from build123d import *

# Parameters (mm, degrees)
SKETCH_1_W      = 8
SKETCH_1_H      = 26
EXTRUDE_1_DEPTH = 525


with BuildPart() as part:
    # 草图1 → 凸台-拉伸1 (new, symmetric)
    with BuildSketch(Plane.XY):
        Polygon((-12, 4.5), (-10, 4.5), (-10, 6.5), (-4, 6.5), (-4, -6.5), (-10, -6.5), (-10, -4.5), (-12, -4.5), (-12, -36.5), (0, -36.5), (0, 36.5), (-12, 36.5), align=None)
        with Locations((-6, -21.5)):
            Rectangle(SKETCH_1_W, SKETCH_1_H, mode=Mode.SUBTRACT)
        with Locations((-6, 21.5)):
            Rectangle(SKETCH_1_W, SKETCH_1_H, mode=Mode.SUBTRACT)
    extrude(amount=EXTRUDE_1_DEPTH, both=True)


solid = part.part
Here's how the part is built. I have some questions about the finished solid (model axes, mm). A direction names the side the tool comes from. Give positions to 0.01 mm unless a question says otherwise; leave off trailing zeros. Order: outer loops, then holes, each group sorted by start corner. A loop starts at its lowest first (then second) coordinate and runs counter-clockwise, first axis right, second up. Notation, with made-up numbers: (-24, 78.25) -> (27, 78.25) arc R30 ccw to (27, 100.25) -> close; hole circle Ø8 at (57.5, 24). An arc over 180 degrees is marked (long way). Use a Markdown table: item, result. Add a question column.
Item 1: Imagine slicing it at C-C on z = 237. Please give me the cut outline in (x, y), plus the area to 3 significant figures.
Item 2: Imagine slicing it at B-B on x = -8. Please give me the cut outline in (y, z).
Item 3: If we mould it in two halves opening along Y, with no side actions, what happens to faces 3 (the face through (-2, 21, 7)), 4 (the face through (-12, 21, 7))? For each: pulls with the +Y half, pulls with the -Y half, needs draft (parallel to the pull), parting line crosses it, or undercut.
Item 4: Imagine slicing it at A-A on y = -17. Please give me the cut outline in (x, z), plus the area to 3 significant figures.
Item 5: Will this pin go through, and if not, where does the flat tip stop? pin 1 (5 mm diameter, centred on y = -6, z = 157.5, fed in from +X).
Item 6: For faces 1 (the face through (-10, -22, 7)), 2 (the face through (0, -1, 7)), which set-ups out of +Z, -Z, +X, -X, +Y, -Y let a thin tool reach every point of the face, with its end or its side?
Item 7: I need wall thicknesses on line 1 (Y direction, x = -9, z = 65); line 2 (X direction, y = 26, z = -202.5); line 3 (X direction, y = -5.5, z = -147.5). Which ranges of each line are inside material? Lowest first, please.
Data:
| question | item | result |
|---|---|---|
| 1 | outline | (-12, -36.5) -> (0, -36.5) -> (0, 36.5) -> (-12, 36.5) -> (-12, 4.5) -> (-10, 4.5) -> (-10, 6.5) -> (-4, 6.5) -> (-4, -6.5) -> (-10, -6.5) -> (-10, -4.5) -> (-12, -4.5) -> close; hole (-10, -34.5) -> (-2, -34.5) -> (-2, -8.5) -> (-10, -8.5) -> close; hole (-10, 8.5) -> (-2, 8.5) -> (-2, 34.5) -> (-10, 34.5) -> close |
| 1 | area | 364 mm² |
| 2 | outline | (-36.5, -525) -> (-34.5, -525) -> (-34.5, 525) -> (-36.5, 525) -> close; (-8.5, -525) -> (-6.5, -525) -> (-6.5, 525) -> (-8.5, 525) -> close; (6.5, -525) -> (8.5, -525) -> (8.5, 525) -> (6.5, 525) -> close; (34.5, -525) -> (36.5, -525) -> (36.5, 525) -> (34.5, 525) -> close |
| 3 | face 3 | undercut |
| 3 | face 4 | needs draft |
| 4 | outline | (-12, -525) -> (-10, -525) -> (-10, 525) -> (-12, 525) -> close; (-2, -525) -> (0, -525) -> (0, 525) -> (-2, 525) -> close |
| 4 | area | 4,200 mm² |
| 5 | pin 1 | stops at x = 0 |
| 6 | face 1 | +Z, -Z |
| 6 | face 2 | +Z, -Z, +X, +Y, -Y |
| 7 | line 1 | y = -36.5 to -34.5, -8.5 to -6.5, 6.5 to 8.5, 34.5 to 36.5 |
| 7 | line 2 | x = -12 to -10, -2 to 0 |
| 7 | line 3 | x = -12 to -10, -4 to 0 |
